```python
from build123d import *

# Parameters (mm, degrees)
SKETCH_1_W                = 75
SKETCH_1_H                = 80
EXTRUDE_1_DEPTH           = 5
CHAMFER_1_SIZE            = 3
HOLE_WIZARD_M5_1_D        = 4.2
HOLE_WIZARD_M5_1_DEPTH    = 12.4
HOLE_WIZARD_M5_1_TIP      = 1.2618073
HOLE_WIZARD_1_D           = 5.5
HOLE_WIZARD_1_CBORE_D     = 10
HOLE_WIZARD_1_CBORE_DEPTH = 5.7
HOLE_WIZARD_2_D           = 4.5
HOLE_WIZARD_2_CBORE_D     = 8
HOLE_WIZARD_2_CBORE_DEPTH = 4.6


with BuildPart() as part:
    # 草图1 → 凸台-拉伸1 (new, symmetric)
    with BuildSketch(Plane(origin=(0, 0, 0), x_dir=(1, 0, 0), z_dir=(0, 1, 0))):
        Rectangle(SKETCH_1_W, SKETCH_1_H)
    extrude(amount=EXTRUDE_1_DEPTH, both=True)

    # 倒角1
    chamfer_1_edges = [part.edges().sort_by_distance(p)[0] for p in [
        (-37.5, 0, 40),
        (-37.5, 0, -40),
    ]]
    chamfer(chamfer_1_edges, length=CHAMFER_1_SIZE)

    # M5 螺纹孔1
    with Locations(Plane(origin=(37.5, 0, 0), x_dir=(0, 0, -1), z_dir=(1, 0, 0))):
        with Locations((-30, 0), (30, 0)):
            Hole(HOLE_WIZARD_M5_1_D / 2, depth=HOLE_WIZARD_M5_1_DEPTH)
            with Locations((0, 0, -(HOLE_WIZARD_M5_1_DEPTH + HOLE_WIZARD_M5_1_TIP / 2))):  # 118° drill point
                Cone(0, HOLE_WIZARD_M5_1_D / 2, HOLE_WIZARD_M5_1_TIP, mode=Mode.SUBTRACT)

    # 打孔尺寸(%根据)内六角圆柱头螺钉的类型1 (through all)
    with Locations(Plane.XZ.offset(5)):
        with Locations((-27.5, -26), (14.5, -26), (14.5, 26), (-27.5, 26)):
            CounterBoreHole(HOLE_WIZARD_1_D / 2, HOLE_WIZARD_1_CBORE_D / 2, HOLE_WIZARD_1_CBORE_DEPTH)

    # 打孔尺寸(%根据)内六角圆柱头螺钉的类型2 (through all)
    with Locations(Plane(origin=(0, 5, 0), x_dir=(1, 0, 0), z_dir=(0, 1, 0))):
        with Locations((-30, 0), (20, 0)):
            CounterBoreHole(HOLE_WIZARD_2_D / 2, HOLE_WIZARD_2_CBORE_D / 2, HOLE_WIZARD_2_CBORE_DEPTH)


solid = part.part
```
CAD build for the part. Positions are in the model's coordinates, mm. A direction names the side the tool comes from. Round coordinates to 2 decimals unless told otherwise and drop trailing zeros. Write each loop counter-clockwise with the first axis right and the second up, starting at its lowest first coordinate (ties: lowest second). Pieces come first, ordered by that corner, then holes. Notation, with made-up numbers: (69.25, -2) - (106.25, -2) arc R29 ccw to (106.25, 26) - close; hole circle Ø6 at (-22, -8). An arc over 180 degrees is marked (long way). Return JSON: item names as keys, results as strings. Group by question number.
Item 1: 3-axis set-ups, long thin cutter, end or side, ignore diameter. For faces 1 (the face through (16.8, 2.7, 2.4)), 2 (the face through (17.247, 2.88, -25.879)), 3 (the face through (-25, 0.7, 24)): which of +Z, -Z, +X, -X, +Y, -Y reach the whole face in a straight line?
Item 2: Band-saw the part on B-B on y = -3.25. List the corners of the cut face in (x, z).
Item 3: Band-saw the part on D-D on y = 3. List the corners of the cut face in (x, z).
Item 4: Mould opens along Y. For faces 4 (the face through (24.057, 0.016, -29.636)), 5 (the face through (22, 0.4, 2)), 6 (the face through (16.807, -2.19, -30.436)) say: +Y half, -Y half, draft (parallel to the pull), parting line (faces both ways), or undercut.
Item 5: Band-saw the part on C-C on z = -26. List the corners of the cut face in (x, y).
Item 6: Band-saw the part on A-A on z = 0. List the corners of the cut face in (x, y), plus the area to 3 significant figures.
Item 7: Flat gauge pins, fed straight in: pin 1 Ø5 at (x, z) = (20, 0) entering from +Y; pin 2 Ø5 at (x, z) = (13, 25) entering from -Y. Where does each tip first touch, or does it go through?
Item 8: Probe probe 1 along Z at (x, y) = (14.5, 3.45); probe 2 along Z at (x, y) = (-27.5, -0.9); probe 3 along Y at (x, z) = (29.5, 30). List the from-to ranges inside material, lowest first.
Resolved:
{
 "1": {"face 1": "+Y", "face 2": "+Y, -Y", "face 3": "-Y"},
 "2": {"outline": "(-37.5, -37) - (-34.5, -40) - (37.5, -40) - (37.5, 40) - (-34.5, 40) - (-37.5, 37) - close; hole circle Ø10 at (-27.5, -26); hole circle Ø10 at (-27.5, 26); hole circle Ø4.5 at (-30, 0); hole circle Ø10 at (14.5, -26); hole circle Ø10 at (14.5, 26); hole circle Ø4.5 at (20, 0)"},
 "3": {"outline": "(-37.5, -37) - (-34.5, -40) - (37.5, -40) - (37.5, 40) - (-34.5, 40) - (-37.5, 37) - close; hole circle Ø8 at (-30, 0); hole circle Ø5.5 at (-27.5, -26); hole circle Ø5.5 at (-27.5, 26); hole circle Ø5.5 at (14.5, -26); hole circle Ø5.5 at (14.5, 26); hole circle Ø8 at (20, 0)"},
 "4": {"face 4": "undercut", "face 5": "+Y half", "face 6": "draft"},
 "5": {"outline": "(-37.5, -5) - (-32.5, -5) - (-32.5, 0.7) - (-30.25, 0.7) - (-30.25, 5) - (-37.5, 5) - close; (-24.75, 0.7) - (-22.5, 0.7) - (-22.5, -5) - (9.5, -5) - (9.5, 0.7) - (11.75, 0.7) - (11.75, 5) - (-24.75, 5) - close; (17.25, 0.7) - (19.5, 0.7) - (19.5, -5) - (37.5, -5) - (37.5, 5) - (17.25, 5) - close"},
 "6": {"outline": "(-37.5, -5) - (-32.25, -5) - (-32.25, 0.4) - (-34, 0.4) - (-34, 5) - (-37.5, 5) - close; (-27.75, -5) - (17.75, -5) - (17.75, 0.4) - (16, 0.4) - (16, 5) - (-26, 5) - (-26, 0.4) - (-27.75, 0.4) - close; (22.25, -5) - (37.5, -5) - (37.5, 5) - (24, 5) - (24, 0.4) - (22.25, 0.4) - close", "area": "628 mm²"},
 "7": {"pin 1": "stops at y = 0.4", "pin 2": "stops at y = 0.7"},
 "8": {"probe 1": "z = -40 to -28.75, -23.25 to 23.25, 28.75 to 40", "probe 2": "z = -40 to -31, -21 to 21, 31 to 40", "probe 3": "y = -5 to -2.1, 2.1 to 5"}
}
